Could you check a few things on this model? Use its own coordinates, in mm. A direction names the side the tool comes from. Give positions to 0.01 mm unless a question says otherwise; leave off trailing zeros. Loops run counter-clockwise (first coordinate to the right, second up) from the corner with the lowest first, then second, coordinate; pieces in that order, holes last. Notation, with made-up numbers: (-6, 16) - (2, 16) arc R21 ccw to (2, 36) - close; hole circle Ø9 at (-6, 57). An arc over 180 degrees is marked (long way). One line per item, written item: value. Start each with the question number.
Q1. I want a section at B-B (x = -8). Please give me the cut outline in (y, z).
Q2. I'm going to push flat-ended pins straight in: P1, Ø6.5, axis at y = 12, z = -8.5, coming from the -X side; P2, Ø10, axis at y = 3.5, z = 5.5, coming from the -X side; P3, Ø4, axis at x = -6.5, y = 9.5, coming from the +Z side. Where does each tip first touch, or does it pass through?
Q3. I want a section at C-C (z = 0). Count the separate pieces of the cut face and the enclosed holes in it, then the cut area to 3 significant figures.
Q4. For faces 5 (the face through (17, 28, -9.75)), 6 (the face through (33.1, 21.37, 3.95)), 7 (the face through (17, 28, 9.75)), 8 (the face through (17.465, 3.301, 6.465)), which set-ups out of +Z, -Z, +X, -X, +Y, -Y let a thin tool reach every point of the face, with its end or its side?
Q5. I want a section at A-A (x = 4.5). Please give me the cut outline in (y, z), then the cut area to 3 significant figures.
Q6. If we mould it in two halves opening along Z, with no side actions, what happens to faces 1 (the face through (17, 9, -6.75)), 2 (the face through (-18.1, 21.37, -3.95)), 3 (the face through (-16.9, 25.059, 3.226)), 4 (the face through (17, 27, -6.75))? For each: released by +Z, released by -Z, zero draft, split by the parting line, or undercut.
Q7. If I drill on line 1 (X direction, y = 2.4, z = 0); line 2 (Z direction, x = 19.5, y = 10.25); line 3 (Y direction, x = 16, z = 1.75), over which ranges is the centre line in solid material (lowest first)? Write a range as from..to.
```python
from build123d import *

# Parameters (mm, degrees)
EXTRUDE_1_DEPTH     = 5
EXTRUDE_START       = -5
EXTRUDE_2_DEPTH     = 5
EXTRUDE_3_DEPTH     = 15
EXTRUDE_4_DEPTH     = 5
SKETCH_6_R          = 2.25
CUT_EXTRUDE_1_DEPTH = 4
SKETCH_7_R          = 2.25
CUT_EXTRUDE_2_DEPTH = 4
SKETCH_8_R          = 3
CUT_EXTRUDE_3_DEPTH = 24.1
CUT_EXTRUDE_START   = -19.1
SKETCH_9_R          = 3
CUT_EXTRUDE_4_DEPTH = 19.1


with BuildPart() as part:
    # 草图1 → 旋转1 (revolve)
    with BuildSketch(Plane.XY, mode=Mode.PRIVATE) as revolve_1_sk:
        Polygon((-19.1, 20), (-19.1, 25.8), (-18.1, 25.8), (-18.1, 24), (-17.1, 24), (-17.1, 25.8), (-13.9, 29), (20, 29), (20, 29.75), (28.15, 29.75), (32.1, 25.8), (32.1, 24), (33.1, 24), (33.1, 25.8), (34.1, 25.8), (34.1, 20), align=None)
    revolve(revolve_1_sk.sketch.rotate(Axis((34.1, 20, 0), (-1, 0, 0)), 270), axis=Axis((34.1, 20, 0), (-1, 0, 0)))

    # 草图2 → 凸台-拉伸1 (add)
    with BuildSketch(Plane(origin=(-10, 0, 0), x_dir=(0, 0, -1), z_dir=(1, 0, 0))):
        with BuildLine():
            Line((-9.75, 13.901844541), (-9.75, 4))
            ThreePointArc((-9.75, 4), (-8.578427125, 1.171572875), (-5.75, 0))
            Line((-5.75, 0), (5.75, 0))
            ThreePointArc((5.75, 0), (8.578427125, 1.171572875), (9.75, 4))
            Line((9.75, 4), (9.75, 13.901844541))
            ThreePointArc((9.75, 13.901844541), (11.5, 20), (9.75, 26.098155459))
            Line((9.75, 26.098155459), (9.75, 29))
            Line((9.75, 29), (6.75, 29))
            Line((6.75, 29), (6.75, 22))
            Line((6.75, 22), (-6.75, 22))
            Line((-6.75, 22), (-6.75, 29))
            Line((-6.75, 29), (-9.75, 29))
            Line((-9.75, 29), (-9.75, 26.098155459))
            ThreePointArc((-9.75, 26.098155459), (-11.5, 20), (-9.75, 13.901844541))
        make_face()
        with BuildLine():
            Line((-5.75, 3), (5.75, 3))
            ThreePointArc((5.75, 3), (6.457106781, 3.292893219), (6.75, 4))
            Line((6.75, 4), (6.75, 20))
            Line((6.75, 20), (-6.75, 20))
            Line((-6.75, 20), (-6.75, 4))
            ThreePointArc((-6.75, 4), (-6.457106781, 3.292893219), (-5.75, 3))
        make_face(mode=Mode.SUBTRACT)
    extrude(amount=EXTRUDE_1_DEPTH)

    # 草图3 → 凸台-拉伸2 (add)
    with BuildSketch(Plane(origin=(20, 0, 0), x_dir=(0, 0, -1), z_dir=(1, 0, 0)).offset(EXTRUDE_START)):
        with BuildLine():
            Line((-9.75, 13.901844541), (-9.75, 4))
            ThreePointArc((-9.75, 4), (-8.578427125, 1.171572875), (-5.75, 0))
            Line((-5.75, 0), (5.75, 0))
            ThreePointArc((5.75, 0), (8.578427125, 1.171572875), (9.75, 4))
            Line((9.75, 4), (9.75, 13.901844541))
            ThreePointArc((9.75, 13.901844541), (11.5, 20), (9.75, 26.098155459))
            Line((9.75, 26.098155459), (9.75, 29))
            Line((9.75, 29), (6.75, 29))
            Line((6.75, 29), (6.75, 22))
            Line((6.75, 22), (-6.75, 22))
            Line((-6.75, 22), (-6.75, 29))
            Line((-6.75, 29), (-9.75, 29))
            Line((-9.75, 29), (-9.75, 26.098155459))
            ThreePointArc((-9.75, 26.098155459), (-11.5, 20), (-9.75, 13.901844541))
        make_face()
        with BuildLine():
            Line((-5.75, 3), (5.75, 3))
            ThreePointArc((5.75, 3), (6.457106781, 3.292893219), (6.75, 4))
            Line((6.75, 4), (6.75, 20))
            Line((6.75, 20), (-6.75, 20))
            Line((-6.75, 20), (-6.75, 4))
            ThreePointArc((-6.75, 4), (-6.457106781, 3.292893219), (-5.75, 3))
        make_face(mode=Mode.SUBTRACT)
    extrude(amount=EXTRUDE_2_DEPTH)

    # 草图4 → 凸台-拉伸3 (add)
    with BuildSketch(Plane(origin=(0, 0, 0), x_dir=(0, 0, -1), z_dir=(1, 0, 0))):
        with BuildLine():
            Line((-5.75, 0), (5.75, 0))
            ThreePointArc((5.75, 0), (8.199489743, 0.83772234), (9.622983346, 3))
            Line((9.622983346, 3), (-9.622983346, 3))
            ThreePointArc((-9.622983346, 3), (-8.199489743, 0.83772234), (-5.75, 0))
        make_face()
    extrude(amount=EXTRUDE_3_DEPTH)

    # 草图5 → 凸台-拉伸4 (add)
    with BuildSketch(Plane(origin=(0, 0, 0), x_dir=(0, 0, -1), z_dir=(1, 0, 0)).offset(EXTRUDE_START)):
        with BuildLine():
            Line((-5.75, 0), (5.75, 0))
            ThreePointArc((5.75, 0), (8.199489743, 0.83772234), (9.622983346, 3))
            Line((9.622983346, 3), (-9.622983346, 3))
            ThreePointArc((-9.622983346, 3), (-8.199489743, 0.83772234), (-5.75, 0))
        make_face()
    extrude(amount=EXTRUDE_4_DEPTH)

    # 草图6 → 切除-拉伸1 (cut)
    with BuildSketch(Plane(origin=(0, 0, 0), x_dir=(1, 0, 0), z_dir=(0, 1, 0))):
        with Locations(Location((0, 0, 0), (0, 0, 270))):
            Circle(SKETCH_6_R)
    extrude(amount=CUT_EXTRUDE_1_DEPTH, mode=Mode.SUBTRACT)

    # 草图7 → 切除-拉伸2 (cut)
    with BuildSketch(Plane(origin=(0, 0, 0), x_dir=(1, 0, 0), z_dir=(0, 1, 0))):
        with Locations(Location((10, 0, 0), (0, 0, 270))):
            Circle(SKETCH_7_R)
    extrude(amount=CUT_EXTRUDE_2_DEPTH, mode=Mode.SUBTRACT)

    # 草图8 → 切除-拉伸3 (cut)
    with BuildSketch(Plane(origin=(34.1, 0, 0), x_dir=(0, 0, -1), z_dir=(1, 0, 0))):
        with Locations((0, 20)):
            Circle(SKETCH_8_R)
    extrude(amount=-CUT_EXTRUDE_3_DEPTH, mode=Mode.SUBTRACT)

    # 草图9 → 切除-拉伸4 (cut)
    with BuildSketch(Plane.ZY.offset(19.1).offset(CUT_EXTRUDE_START)):
        with Locations(Location((0, 20, 0), (0, 0, 180))):
            Circle(SKETCH_9_R)
    extrude(amount=CUT_EXTRUDE_4_DEPTH, mode=Mode.SUBTRACT)


solid = part.part
```
Worked answers:
1. outline: (0, -5.75) arc R4 ccw to (4, -9.75) - (13.9, -9.75) arc R11.5 ccw to (26.1, -9.75) - (29, -9.75) - (29, -6.75) - (25.95, -6.75) arc R9 ccw to (25.95, 6.75) - (29, 6.75) - (29, 9.75) - (26.1, 9.75) arc R11.5 ccw to (13.9, 9.75) - (4, 9.75) arc R4 ccw to (0, 5.75) - close; hole (3, -5.75) arc R1 ccw to (4, -6.75) - (14.05, -6.75) arc R9 cw to (14.05, 6.75) - (4, 6.75) arc R1 ccw to (3, 5.75) - close; hole circle Ø6 at (20, 0)
2. P1: stops at x = -14.48
2. P2: stops at x = -10
2. P3: stops at z = 9.75
3. separate pieces: 4
3. enclosed holes: 0
3. area: 721 mm²
4. face 5: -Z, +X, -X, +Y
4. face 6: none
4. face 7: +Z, +X, -X, +Y
4. face 8: +X, -X
5. outline: (0, -5.75) arc R4 ccw to (3, -9.62) - (3, 9.62) arc R4 ccw to (0, 5.75) - close; circle Ø18 at (20, 0)
5. area: 306 mm²
6. face 1: undercut
6. face 2: zero draft
6. face 3: split by the parting line
6. face 4: undercut
7. line 1: x = -10..-2.25, 2.25..7.75, 12.25..20
7. line 2: z = -9.75..-6.75, 6.75..9.75
7. line 3: y = 0..3, 11.17..17.56, 22.44..28.83
